Could you check a few things on this model? Use its own coordinates, in mm. A direction names the side the tool comes from. Coordinates: 2 decimals unless noted, no trailing zeros. Loops run counter-clockwise (first coordinate to the right, second up) from the corner with the lowest first, then second, coordinate; pieces in that order, holes last. Notation, with made-up numbers: (29, 41) - (70, 41) arc R25 cw to (70, 69) - close; hole circle Ø5 at (84.5, -28). An arc over 180 degrees is marked (long way). Use CSV: the item, a comma, the result in double quotes.
from build123d import *


with BuildPart() as part:
    # Sketch1 → Revolve1 (revolve)
    with BuildSketch(Plane(origin=(0, 0, 0), x_dir=(1, 0, 0), z_dir=(0, 1, 0)), mode=Mode.PRIVATE) as revolve1_sk:
        Polygon((0, 150), (0, 163), (14, 163), (14, 177), (0, 177), (0, 189), (14, 189), (14, 203), (0, 203), (0, 219.5), (45, 219.5), (45, 227.5), (59, 227.5), (59, 219.5), (74, 219.5), (74, 200), (30, 200), (30, 150), align=None)
    revolve(revolve1_sk.sketch.rotate(Axis((0, 0, 0), (1, 0, 0)), 180), axis=Axis((0, 0, 0), (1, 0, 0)))


solid = part.part
(1) Please list where these lines run through material, in increasing order: line 1 (Y direction, x = 8, z = 0); line 2 (Y direction, x = 5, z = -34.5); line 3 (X direction, y = -110.5, z = -131.5).
Computed:
line 1,"y = -219.5 to -203, -189 to -177, -163 to -150, 150 to 163, 177 to 189, 203 to 219.5"
line 2,"y = -216.77 to -200.05, -185.82 to -173.61, -159.31 to -145.98, 145.98 to 159.31, 173.61 to 185.82, 200.05 to 216.77"
line 3,"x = 14 to 30"
(2) Thinking about a two-plate mould opening in Z: for faces 4 (the face through (45, -186, 119)), 5 (the face through (6.902, -60.976, 193.626)), 6 (the face through (22.82, 214.28, -47.58)), which applies, +Z half, -Z half, draft (parallel to the pull), parting line (faces both ways), or undercut?
Computed:
face 4,"draft"
face 5,"undercut"
face 6,"parting line"
(3) Suppose I cut it at A-A (x = 7). Write out the boundary of the cut face in (y, z), plus the area to 3 significant figures.
Computed:
outline,"circle Ø439 at (0, 0); circle Ø378 at (0, 0); circle Ø326 at (0, 0); hole circle Ø406 at (0, 0); hole circle Ø354 at (0, 0); hole circle Ø300 at (0, 0)"
area,"48,500 mm²"
(4) Which directions (+Z, -Z, +X, -X, +Y, -Y) give clear straight access to the entire face, cutting with the end or side of a thin tool? Please do faces 1 (the face through (0, 64, -194)), 2 (the face through (59, -186, -119)), 3 (the face through (7.1, 62.43, 150.57)).
Computed:
face 1,"+Z, -Z, -X, +Y, -Y"
face 2,"+X"
face 3,"-X"
(5) Will these pins go through, and if not, where does the flat tip stop? pin 1 (8 mm diameter, centred on x = 38, y = 102.5, fed in from +Z); pin 2 (3 mm diameter, centred on x = 12.5, z = -34.5, fed in from -Y); pin 3 (4 mm diameter, centred on y = 40, z = 165, fed in from -X).
Computed:
pin 1,"stops at z = 196.16"
pin 2,"stops at y = -217.01"
pin 3,"stops at x = 14"
